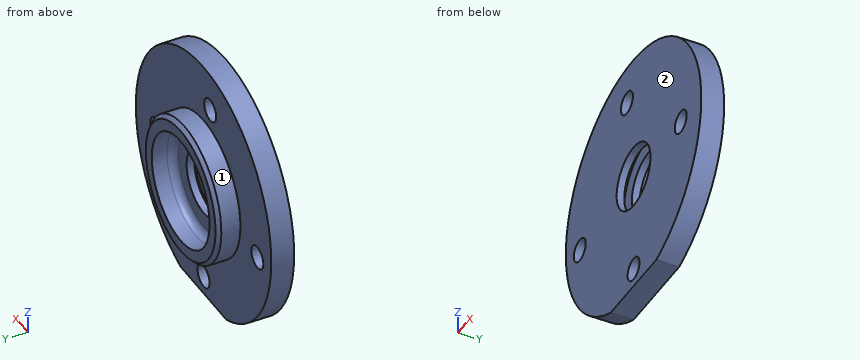
from build123d import *

# Parameters (mm, degrees)
SKETCH1_R           = 34
BOSS_EXTRUDE1_DEPTH = 6
SKETCH2_R           = 18.5
BOSS_EXTRUDE2_DEPTH = 6
SKETCH3_R           = 14.5
CUT_EXTRUDE1_DEPTH  = 6
SKETCH4_R           = 8.5
CUT_EXTRUDE2_DEPTH  = 2
SKETCH5_R           = 12.5
CUT_EXTRUDE3_DEPTH  = 2
SKETCH6_R           = 8.5
CUT_EXTRUDE4_DEPTH  = 2
CHAMFER1_SIZE       = 1
FILLET1_R           = 2
SKETCH7_W           = 39.246802542
SKETCH7_H           = 4
CUT_EXTRUDE5_DEPTH  = 23
SKETCH8_R           = 3
CUT_EXTRUDE6_DEPTH  = 80


with BuildPart() as part:
    # Sketch1 → Boss-Extrude1 (new body)
    with BuildSketch(Plane(origin=(0, 0, 0), x_dir=(1, 0, 0), z_dir=(0, 1, 0))):
        with Locations(Location((0, 0, 0), (0, 0, 270))):
            Circle(SKETCH1_R)
    extrude(amount=BOSS_EXTRUDE1_DEPTH)

    # Sketch2 → Boss-Extrude2 (add)
    with BuildSketch(Plane(origin=(0, 6, 0), x_dir=(1, 0, 0), z_dir=(0, 1, 0))):
        with Locations(Location((0, 0, 0), (0, 0, 270))):
            Circle(SKETCH2_R)
    extrude(amount=BOSS_EXTRUDE2_DEPTH)

    # Sketch3 → Cut-Extrude1 (cut)
    with BuildSketch(Plane(origin=(0, 12, 0), x_dir=(1, 0, 0), z_dir=(0, 1, 0))):
        with Locations(Location((0, 0, 0), (0, 0, 270))):
            Circle(SKETCH3_R)
    extrude(amount=-CUT_EXTRUDE1_DEPTH, mode=Mode.SUBTRACT)

    # Sketch4 → Cut-Extrude2 (cut)
    with BuildSketch(Plane(origin=(0, 6, 0), x_dir=(1, 0, 0), z_dir=(0, 1, 0))):
        with Locations(Location((0, 0, 0), (0, 0, 270))):
            Circle(SKETCH4_R)
    extrude(amount=-CUT_EXTRUDE2_DEPTH, mode=Mode.SUBTRACT)

    # Sketch5 → Cut-Extrude3 (cut)
    with BuildSketch(Plane(origin=(0, 4, 0), x_dir=(1, 0, 0), z_dir=(0, 1, 0))):
        with Locations(Location((0, 0, 0), (0, 0, 270))):
            Circle(SKETCH5_R)
    extrude(amount=-CUT_EXTRUDE3_DEPTH, mode=Mode.SUBTRACT)

    # Sketch6 → Cut-Extrude4 (cut)
    with BuildSketch(Plane(origin=(0, 2, 0), x_dir=(1, 0, 0), z_dir=(0, 1, 0))):
        with Locations(Location((0, 0, 0), (0, 0, 270))):
            Circle(SKETCH6_R)
    extrude(amount=-CUT_EXTRUDE4_DEPTH, mode=Mode.SUBTRACT)

    # Chamfer1
    chamfer1_edges = [part.edges().sort_by_distance(p)[0] for p in [
        (0, 12, -18.5),
    ]]
    chamfer(chamfer1_edges, length=CHAMFER1_SIZE)

    # Fillet1
    fillet1_edges = [part.edges().sort_by_distance(p)[0] for p in [
        (0, 6, -14.5),
    ]]
    fillet(fillet1_edges, radius=FILLET1_R)

    # Sketch7 → Cut-Extrude5 (cut)
    with BuildSketch(Plane(origin=(0, 6, 0), x_dir=(1, 0, 0), z_dir=(0, 1, 0))):
        with Locations((0, 34)):
            Rectangle(SKETCH7_W, SKETCH7_H)
    extrude(amount=-CUT_EXTRUDE5_DEPTH, mode=Mode.SUBTRACT)

    # Sketch8 → Cut-Extrude6 (cut)
    with BuildSketch(Plane(origin=(0, 6, 0), x_dir=(1, 0, 0), z_dir=(0, 1, 0))):
        with Locations(Location((0, 27, 0), (0, 0, 270))):
            Circle(SKETCH8_R)
        with Locations(Location((23.68, 0, 0), (0, 0, 270))):
            Circle(SKETCH8_R)
        with Locations(Location((-3.32, -23.68, 0), (0, 0, 270))):
            Circle(SKETCH8_R)
        with Locations(Location((-27, 3.32, 0), (0, 0, 270))):
            Circle(SKETCH8_R)
    extrude(amount=-CUT_EXTRUDE6_DEPTH, mode=Mode.SUBTRACT)


solid = part.part
CAD build for the part. Positions are in the model's coordinates, mm. Face numbers are marked on the shaded views. A direction names the side the tool comes from. Round coordinates to 2 decimals unless told otherwise and drop trailing zeros. Loops run counter-clockwise (first coordinate to the right, second up) from the corner with the lowest first, then second, coordinate; pieces in that order, holes last.
(1) Cut at B-B (x = -27). Give the cut face in (y, z).
(2) Drop flat-ended pins along their axis: pin 1 (3.5 mm diameter, centred on x = 23.68, z = 0, fed in from -Y); pin 2 (5 mm diameter, centred on x = -21, y = 7.5, fed in from +Z); pin 3 (7.5 mm diameter, centred on x = -2.5, z = 5, fed in from +Y); pin 4 (6 mm diameter, centred on y = 2, z = -10, fed in from -X). Give the stop position or say it passes through.
(3) Cut at D-D (z = -23). Give the cut face in (x, y).
(4) Cut at C-C (y = 7). Give the cut face in (x, z), plus the area to 3 significant figures.
(5) Wall check: line 1 along Y through (x, z) = (-12, -23); line 2 along Y through (x, z) = (3, -9.5); line 3 along Z through (x, y) = (-27.5, 4.25). Give the ranges that are in metal, low to high.
(6) Which spindle directions (+Z, -Z, +X, -X, +Y, -Y) get a long thin tool onto all of the face, cutting with end or side? Do the marked faces 1 and 2. Say none if no direction does.
(7) Cut at A-A (x = 23.68). Give the cut face in (y, z).
Findings below:
1. outline: (0, -20.66) - (6, -20.66) - (6, -6.32) - (0, -6.32) - close; (0, -0.32) - (6, -0.32) - (6, 20.66) - (0, 20.66) - close
2. pin 1: passes through
2. pin 2: stops at z = 28.2
2. pin 3: stops at y = 6
2. pin 4: stops at x = -33.27
3. outline: (-25.04, 0) - (25.04, 0) - (25.04, 6) - (-25.04, 6) - close
4. outline: circle Ø37 at (0, 0); hole circle Ø28.46 at (0, 0)
4. area: 439 mm2
5. line 1: y = 0 to 6
5. line 2: y = 0 to 2, 4 to 6
5. line 3: z = -19.99 to -6.28, -0.36 to 19.99
6. face 1: +Y
6. face 2: +Z, -Z, +X, -X, -Y
7. outline: (0, -24.4) - (6, -24.4) - (6, -3) - (0, -3) - close; (0, 3) - (6, 3) - (6, 24.4) - (0, 24.4) - close
